from build123d import *

# Parameters (mm, degrees)
SKETCH1_W              = 230
SKETCH1_H              = 110
BOSS_EXTRUDE1_DEPTH    = 15
M12_TAPPED_HOLE2_D     = 10.2
M12_TAPPED_HOLE2_DEPTH = 29.25
M12_TAPPED_HOLE2_TIP   = 3.064389157


with BuildPart() as part:
    # Sketch1 → Boss-Extrude1 (new body)
    with BuildSketch(Plane.XY):
        Rectangle(SKETCH1_W, SKETCH1_H)
    extrude(amount=BOSS_EXTRUDE1_DEPTH)

    # M12 Tapped Hole2
    with Locations(Plane.XY.offset(15)):
        with Locations((-97.5, -35), (97.5, -35), (0, 35), (0, -35)):
            Hole(M12_TAPPED_HOLE2_D / 2, depth=M12_TAPPED_HOLE2_DEPTH)
            with Locations((0, 0, -(M12_TAPPED_HOLE2_DEPTH + M12_TAPPED_HOLE2_TIP / 2))):  # 118° drill point
                Cone(0, M12_TAPPED_HOLE2_D / 2, M12_TAPPED_HOLE2_TIP, mode=Mode.SUBTRACT)


solid = part.part
The listing builds one solid part. Answer for the finished solid, in the listing's coordinates (mm). Give positions to 0.01 mm unless a question says otherwise; leave off trailing zeros. Write each loop counter-clockwise with the first axis right and the second up, starting at its lowest first coordinate (ties: lowest second). Pieces come first, ordered by that corner, then holes. Notation, with made-up numbers: (86.25, 87.5) -> (101.25, 87.5) arc R13 cw to (101.25, 93.5) -> close; hole circle Ø10 at (6, 32). An arc over 180 degrees is marked (long way). Use a Markdown table: item, result.
(1) A flat-ended cylindrical pin translates along its axis: P1, Ø8, axis at x = -97.5, y = -35, coming from the -Z side. Find the tip coordinate at first contact, or state that the pin passes through.
Return value:
| item | result |
|---|---|
| P1 | through |
(2) Find the intervals of material crossed by probe 1 along Y at (x, z) = (0, 8.75); probe 2 along Y at (x, z) = (-97.5, 7.5); probe 3 along X at (y, z) = (-38, 1), in increasing order. Write a range as from..to.
Return value:
| item | result |
|---|---|
| probe 1 | -55..-40.1, -29.9..29.9, 40.1..55 |
| probe 2 | -55..-40.1, -29.9..55 |
| probe 3 | -115..-101.62, -93.38..-4.12, 4.12..93.38, 101.62..115 |
(3) Section B-B, the plane x = 97.5 is taken. Determine the outline of the cut face in (y, z).
Return value:
| item | result |
|---|---|
| outline | (-55, 0) -> (-40.1, 0) -> (-40.1, 15) -> (-55, 15) -> close; (-29.9, 0) -> (55, 0) -> (55, 15) -> (-29.9, 15) -> close |
(4) Determine the mould class of faces 1 (the flat face through (-2, 1, 0)), 2 (the flat face through (-115, -1, 7)), 3 (the cylindrical face through (-92.405, -34.776, 7.395)) for opening direction X: released by +X, released by -X, zero draft, split by the parting line, or undercut.
Return value:
| item | result |
|---|---|
| face 1 | zero draft |
| face 2 | released by -X |
| face 3 | undercut |
(5) Section C-C, the plane x = 0 is taken. Determine the outline of the cut face in (y, z).
Return value:
| item | result |
|---|---|
| outline | (-55, 0) -> (-40.1, 0) -> (-40.1, 15) -> (-55, 15) -> close; (-29.9, 0) -> (29.9, 0) -> (29.9, 15) -> (-29.9, 15) -> close; (40.1, 0) -> (55, 0) -> (55, 15) -> (40.1, 15) -> close |
(6) Section A-A, the plane y = 35 is taken. Determine the outline of the cut face in (x, z).
Return value:
| item | result |
|---|---|
| outline | (-115, 0) -> (-5.1, 0) -> (-5.1, 15) -> (-115, 15) -> close; (5.1, 0) -> (115, 0) -> (115, 15) -> (5.1, 15) -> close |
